The model under review builds one solid part; all positions refer to its coordinate system, in mm. A direction names the side the tool comes from. Round coordinates to 2 decimals unless told otherwise and drop trailing zeros. Write each loop counter-clockwise with the first axis right and the second up, starting at its lowest first coordinate (ties: lowest second). Pieces come first, ordered by that corner, then holes. Notation, with made-up numbers: (-1.75, 33) -> (40.25, 33) arc R28 cw to (40.25, 69) -> close; hole circle Ø2 at (-13.75, -19). An arc over 180 degrees is marked (long way). Use CSV: the item, a comma, the result in double quotes. Start each with the question number.
1) Take a section at D-D, the plane y = 43.5. Give the boundary of the cut face in (x, z).
2) Take a section at C-C, the plane z = -8. Give the boundary of the cut face in (x, y).
3) Take a section at B-B, the plane y = 28.5. Give the boundary of the cut face in (x, z), then the cut area to 3 significant figures.
4) Machinability: for faces 4 (the face through (-47.73, 55.24, 16.2)), 5 (the face through (-45.4, 30.4, 12.5)), which of the approach directions +Z, -Z, +X, -X, +Y, -Y give a long, thin tool a straight path to every point of the face, cutting with its end or side? Answer none if there is none.
5) Mouldability with a two-part tool opening along Z and no side actions: class faces 1 (the face through (71, 0, 0)), 2 (the face through (-3, 24, -20)), 3 (the face through (-45.4, 30.4, -12.5)) as released by +Z, released by -Z, zero draft, split by the parting line, or undercut.
6) Wall thickness on probe 1 along Z at (x, y) = (-39.5, 13); probe 2 along X at (y, z) = (3, 8); probe 3 along Y at (x, z) = (79, -13): over which ranges is each line inside the solid? List them lowest first. Write a range as [from, to].
7) Take a section at A-A, the plane z = 17. Give the boundary of the cut face in (x, y), then the cut area to 3 significant figures.
8) For pin 1 Ø6.5 at (x, y) = (-49.88, 51.87) entering from +Z; pin 2 Ø6 at (x, z) = (5, -1.5) entering from +Y; pin 3 Ø7.5 at (y, z) = (32.5, 4.5) entering from -X; pin 4 Ø1.5 at (x, z) = (25.5, -7) entering from -Y, all flat-tipped, find the tip position at first contact; note any pin that passes through.
from build123d import *

# Parameters (mm, degrees)
JAW_PROFILE_SKETCH_R        = 4
JAW_PLATE_40MM_DEPTH        = 20
CLEVIS_SLOT_25MM_DEPTH      = 107.52257834
CLEVIS_SLOT_25MM_DEPTH_BACK = 107.52257834
CLEVIS_SLOT_SKETCH_W        = 50
CLEVIS_SLOT_SKETCH_H        = 25


with BuildPart() as part:
    # Jaw Profile Sketch → Jaw Plate 40mm (new, symmetric)
    with BuildSketch(Plane.XY):
        with BuildLine():
            Line((-39.194156399, 0), (0, 0))
            ThreePointArc((0, 0), (30.805843601, 13), (61.611687203, 0))
            Line((61.611687203, 0), (80.805843601, 0))
            ThreePointArc((80.805843601, 0), (85.299901044, 2.808323085), (84.745652382, 8.07862092))
            Line((84.745652382, 8.07862092), (80.057169629, 14.07862092))
            ThreePointArc((80.057169629, 14.07862092), (79.030253505, 15.063872091), (77.767360848, 15.71990466))
            Line((77.767360848, 15.71990466), (-47.244156399, 59.421847456))
            ThreePointArc((-47.244156399, 59.421847456), (-55.398946719, 57.665436802), (-57.55764481, 49.607794087))
            Line((-57.55764481, 49.607794087), (-43.990086656, 3.586121305))
            ThreePointArc((-43.990086656, 3.586121305), (-42.188368025, 0.995665256), (-39.194156399, 0))
        make_face()
        with Locations((-49.884156399, 51.87)):
            Circle(JAW_PROFILE_SKETCH_R, mode=Mode.SUBTRACT)
        with Locations((-42.554156399, 27)):
            Circle(JAW_PROFILE_SKETCH_R, mode=Mode.SUBTRACT)
    extrude(amount=JAW_PLATE_40MM_DEPTH, both=True)

    # Clevis Slot Sketch → Clevis Slot 25mm (cut, two sides: drawn at the far end of the back side and taken through both)
    with BuildSketch(Plane.XZ.offset(-CLEVIS_SLOT_25MM_DEPTH_BACK)):
        with Locations((-57.55764481, 0)):
            Rectangle(CLEVIS_SLOT_SKETCH_W, CLEVIS_SLOT_SKETCH_H)
    extrude(amount=CLEVIS_SLOT_25MM_DEPTH + CLEVIS_SLOT_25MM_DEPTH_BACK, mode=Mode.SUBTRACT)


solid = part.part
Values found:
1,outline,"(-55.76, -20) -> (-1.7, -20) -> (-1.7, 20) -> (-55.76, 20) -> (-55.76, 12.5) -> (-32.56, 12.5) -> (-32.56, -12.5) -> (-55.76, -12.5) -> close"
2,outline,"(-32.56, 0) -> (0, 0) arc R43 cw to (61.61, 0) -> (80.81, 0) arc R5 ccw to (84.75, 8.08) -> (80.06, 14.08) arc R5 ccw to (77.77, 15.72) -> (-32.56, 54.29) -> close"
3,outline,"(-51.33, -20) -> (-46.26, -20) -> (-46.26, -12.5) -> (-51.33, -12.5) -> close; (-51.33, 12.5) -> (-46.26, 12.5) -> (-46.26, 20) -> (-51.33, 20) -> close; (-38.85, -20) -> (41.21, -20) -> (41.21, 20) -> (-38.85, 20) -> (-38.85, 12.5) -> (-32.56, 12.5) -> (-32.56, -12.5) -> (-38.85, -12.5) -> close"
3,area,"3,120 mm²"
4,face 4,"+Z, -Z"
4,face 5,"-X, +Y, -Y"
5,face 1,"zero draft"
5,face 2,"released by -Z"
5,face 3,"undercut"
6,probe 1,"[-20, -12.5], [12.5, 20]"
6,probe 2,"[-32.56, 3.24], [58.37, 85.39]"
6,probe 3,"[0, 15.09]"
7,outline,"(-57.56, 49.61) -> (-43.99, 3.59) arc R5 ccw to (-39.19, 0) -> (0, 0) arc R43 cw to (61.61, 0) -> (80.81, 0) arc R5 ccw to (84.75, 8.08) -> (80.06, 14.08) arc R5 ccw to (77.77, 15.72) -> (-47.24, 59.42) arc R8 ccw to start; hole circle Ø8 at (-49.88, 51.87); hole circle Ø8 at (-42.55, 27)"
7,area,"4,370 mm²"
8,pin 1,"through"
8,pin 2,"y = 42.21"
8,pin 3,"x = -32.56"
8,pin 4,"y = 12.57"
